```python
from build123d import *

# Parameters (mm, degrees)
CUT_EXTRUDE1_REACH = 663.648
SKETCH2_R          = 20
CUT_EXTRUDE2_DEPTH = 30
CUT_EXTRUDE3_DEPTH = 30


with BuildPart() as part:
    # Sketch1 → Revolve1 (revolve)
    with BuildSketch(Plane.XY, mode=Mode.PRIVATE) as revolve1_sk:
        Polygon((0, 0), (25, 0), (25, 330), (33, 330), (33, 340), (25, 340), (25, 585.119663834), (25, 619.032357738), (25, 660), (0, 660), align=None)
    revolve(revolve1_sk.sketch.rotate(Axis((0, 660, 0), (0, -1, 0)), 180), axis=Axis((0, 660, 0), (0, -1, 0)))

    # Sketch2 → Cut-Extrude1 (cut, up to next)
    with BuildSketch(Plane(origin=(0, 660, 0), x_dir=(1, 0, 0), z_dir=(0, 1, 0)), mode=Mode.PRIVATE) as cut_extrude1_sk1:
        with Locations(Location((0, 0, 0), (0, 0, 180))):
            Circle(SKETCH2_R)
    cut_extrude1_tool1 = extrude(cut_extrude1_sk1.sketch, amount=-CUT_EXTRUDE1_REACH, mode=Mode.PRIVATE) & part.part
    add(cut_extrude1_tool1.solids().sort_by_distance((0, 660, 0))[0], mode=Mode.SUBTRACT)

    # Sketch3 → Cut-Extrude2 (cut)
    with BuildSketch(Plane(origin=(0, 660, 0), x_dir=(1, 0, 0), z_dir=(0, 1, 0))):
        with BuildLine():
            Line((0, -43.201505936), (0, 0))
            Line((0, 0), (43.201505936, 0))
            ThreePointArc((43.201505936, 0), (30.548077804, -30.548077804), (0, -43.201505936))
        make_face()
    extrude(amount=-CUT_EXTRUDE2_DEPTH, mode=Mode.SUBTRACT)

    # Sketch4 → Cut-Extrude3 (cut)
    with BuildSketch(Plane.XZ):
        with BuildLine():
            Line((51.068202024, 0), (0, 0))
            Line((0, 0), (0, 51.068202024))
            ThreePointArc((0, 51.068202024), (36.110671954, 36.110671954), (51.068202024, 0))
        make_face()
    extrude(amount=-CUT_EXTRUDE3_DEPTH, mode=Mode.SUBTRACT)


solid = part.part
```
Here's how the part is built. I have some questions about the finished solid (model axes, mm). A direction names the side the tool comes from. Round coordinates to 2 decimals unless told otherwise and drop trailing zeros. Order: outer loops, then holes, each group sorted by start corner. A loop starts at its lowest first (then second) coordinate and runs counter-clockwise, first axis right, second up. Notation, with made-up numbers: (-27.5, 63) -> (29.5, 63) arc R25 ccw to (29.5, 97) -> close; hole circle Ø9 at (-13, 52). An arc over 180 degrees is marked (long way). Use a Markdown table: item, result. Add a question column.
(1) Suppose I cut it at C-C, the plane y = 107. Please give me the cut outline in (x, z), and give its area (3 significant figures).
(2) For pin 1 Ø8 at (y, z) = (75.5, -25) entering from +X; pin 2 Ø5.5 at (x, y) = (23.5, 14.5) entering from +Z; pin 3 Ø3 at (y, z) = (455.5, 12) entering from -X, each with a flat end and sliding along its axis, tell me the tip position at first contact or that it passes through.
(3) Suppose I cut it at A-A, the plane x = 14. Please give me the cut outline in (y, z).
(4) For faces 1 (the face through (5, 340, -25)), 2 (the face through (-13.44, 167.31, -21.08)), 3 (the face through (14.4, 630, 14.3)), which set-ups out of +Z, -Z, +X, -X, +Y, -Y let a thin tool reach every point of the face, with its end or its side?
(5) If we mould it in two halves opening along Z, with no side actions, what happens to faces 4 (the face through (19.98, 334.62, 0.88)), 5 (the face through (-13.44, 502.24, -21.08)), 6 (the face through (-5, 330, -25))? For each: released by +Z, released by -Z, zero draft, split by the parting line, or undercut.
(6) Suppose I cut it at B-B, the plane z = -7.5. Please give me the cut outline in (x, y).
(7) I need wall thicknesses on line 1 along Z through (x, y) = (0, 392); line 2 along X through (y, z) = (264, -1); line 3 along Y through (x, z) = (-18, -20). Which ranges of each line are inside material? Lowest first, please.
Verdict:
| question | item | result |
|---|---|---|
| 1 | outline | circle Ø50 at (0, 0); hole circle Ø40 at (0, 0) |
| 1 | area | 707 mm2 |
| 2 | pin 1 | x = 13.56 |
| 2 | pin 2 | z = 0 |
| 2 | pin 3 | x = -22.69 |
| 3 | outline | (0, -20.71) -> (330, -20.71) -> (330, -29.88) -> (340, -29.88) -> (340, -20.71) -> (660, -20.71) -> (660, -14.28) -> (0, -14.28) -> close; (30, 14.28) -> (630, 14.28) -> (630, 20.71) -> (340, 20.71) -> (340, 29.88) -> (330, 29.88) -> (330, 20.71) -> (30, 20.71) -> close |
| 4 | face 1 | +Y |
| 4 | face 2 | -Y |
| 4 | face 3 | +Z, +X, +Y |
| 5 | face 4 | undercut |
| 5 | face 5 | split by the parting line |
| 5 | face 6 | zero draft |
| 6 | outline | (-32.14, 330) -> (-23.85, 330) -> (-23.85, 0) -> (-18.54, 0) -> (-18.54, 660) -> (-23.85, 660) -> (-23.85, 340) -> (-32.14, 340) -> close; (18.54, 0) -> (23.85, 0) -> (23.85, 330) -> (32.14, 330) -> (32.14, 340) -> (23.85, 340) -> (23.85, 660) -> (18.54, 660) -> close |
| 7 | line 1 | -25 to -20, 20 to 25 |
| 7 | line 2 | -24.98 to -19.97, 19.97 to 24.98 |
| 7 | line 3 | 330 to 340 |
